Could you check a few things on this model? Use its own coordinates, in mm. A direction names the side the tool comes from. Give positions to 0.01 mm unless a question says otherwise; leave off trailing zeros. Order: outer loops, then holes, each group sorted by start corner. A loop starts at its lowest first (then second) coordinate and runs counter-clockwise, first axis right, second up. Notation, with made-up numbers: M 73,7.5 L 79,7.5 A15 ccw 79,25.5 Z; hole C 32,51.5 d6. An arc over 180 degrees is marked long. Use a Markdown table: item, result. Add a question column.
Item 1: Suppose I cut it at A-A on z = 28.5. Write out the boundary of the cut face in (x, y), plus the area to 3 significant figures.
Item 2: Suppose I cut it at B-B on x = 62. Count the separate pieces of the cut face and the enclosed holes in it, plus the area to 3 significant figures.
Item 3: If I drill on L1, parallel to Y at x = 60, z = 16; L2, parallel to X at y = 55.5, z = 36.5; L3, parallel to Y at x = 11.5, z = 43, over which ranges is the centre line in solid material (lowest first)? Write a range as from..to.
Item 4: If we mould it in two halves opening along X, with no side actions, what happens to faces 4 (the face through (2.85, 66.99, 5.07)), 5 (the face through (54.5, 65.1, 52.5)), 6 (the face through (65, 58, 55))? For each: released by +X, released by -X, zero draft, split by the parting line, or undercut.
Item 5: Suppose I cut it at C-C on x = 54. Write out the boundary of the cut face in (y, z), plus the area to 3 significant figures.
Item 6: I'm going to push flat-ended pins straight in: pin 1 Ø7.5 at (x, y) = (13, 11.5) entering from +Z; pin 2 Ø7.5 at (x, y) = (61, 9.5) entering from +Z; pin 3 Ø6 at (x, z) = (18.5, 53.5) entering from +Y; pin 4 Ø1.5 at (x, z) = (13, 33.5) entering from +Y. Where does each tip first touch, or does it pass through?
Item 7: For faces 1 (the face through (54.048, 5.436, 52.465)), 2 (the face through (27, 43, 40)), 3 (the face through (70, 35, 5)), which set-ups out of +Z, -Z, +X, -X, +Y, -Y let a thin tool reach every point of the face, with its end or its side?
from build123d import *

# Parameters (mm, degrees)
BASE_PLATE_SKETCH_W             = 70
BASE_PLATE_SKETCH_H             = 70
BASE_PLATE_DEPTH                = 10
CORNER_POSTS_SKETCH_R           = 7.5
CORNER_POSTS_4X_DEPTH           = 30
TOP_PLATE_SKETCH_W              = 70
TOP_PLATE_SKETCH_H              = 70
TOP_PLATE_DEPTH                 = 10
POST_BOSSES_SKETCH_R            = 7.5
POST_BOSSES_SKETCH_R_2          = 5
POST_BOSSES_4X_DEPTH            = 5
CENTRE_BOSS_SKETCH_R            = 15
CENTRE_BOSS_SKETCH_R_2          = 11
CENTRE_BOSS_30_DEPTH            = 20
CENTRE_BORE_SKETCH_R            = 11
CENTRE_BORE_CUT_DEPTH           = 111.905365064
POST_HOLES_SKETCH_R             = 5
POST_HOLES_4X_DEPTH             = 111.905365064
TOP_PLATE_CORNER_FILLETS_R10_R  = 10
BASE_PLATE_CORNER_FILLETS_R10_R = 10


with BuildPart() as part:
    # Base Plate Sketch → Base Plate (new body)
    with BuildSketch(Plane.XY):
        with Locations((35, 35)):
            Rectangle(BASE_PLATE_SKETCH_W, BASE_PLATE_SKETCH_H)
    extrude(amount=BASE_PLATE_DEPTH)

    # Corner Posts Sketch → Corner Posts 4x (add)
    with BuildSketch(Plane.XY.offset(10)):
        with Locations((10, 10)):
            Circle(CORNER_POSTS_SKETCH_R)
        with Locations((60, 10)):
            Circle(CORNER_POSTS_SKETCH_R)
        with Locations((60, 60)):
            Circle(CORNER_POSTS_SKETCH_R)
        with Locations((10, 60)):
            Circle(CORNER_POSTS_SKETCH_R)
    extrude(amount=CORNER_POSTS_4X_DEPTH)

    # Top Plate Sketch → Top Plate (add)
    with BuildSketch(Plane.XY.offset(40)):
        with Locations((35, 35)):
            Rectangle(TOP_PLATE_SKETCH_W, TOP_PLATE_SKETCH_H)
    extrude(amount=TOP_PLATE_DEPTH)

    # Post Bosses Sketch → Post Bosses 4x (add)
    # profile 1 of 4: a face of its own
    with BuildSketch(Plane.XY.offset(50)):
        with Locations((10, 60)):
            Circle(POST_BOSSES_SKETCH_R)
        with Locations((10, 60)):
            Circle(POST_BOSSES_SKETCH_R_2, mode=Mode.SUBTRACT)
    # profile 2 of 4: a face of its own
    with BuildSketch(Plane.XY.offset(50)):
        with Locations((60, 60)):
            Circle(POST_BOSSES_SKETCH_R)
        with Locations((60, 60)):
            Circle(POST_BOSSES_SKETCH_R_2, mode=Mode.SUBTRACT)
    # profile 3 of 4: a face of its own
    with BuildSketch(Plane.XY.offset(50)):
        with Locations((10, 10)):
            Circle(POST_BOSSES_SKETCH_R)
        with Locations((10, 10)):
            Circle(POST_BOSSES_SKETCH_R_2, mode=Mode.SUBTRACT)
    # profile 4 of 4: a face of its own
    with BuildSketch(Plane.XY.offset(50)):
        with Locations((60, 10)):
            Circle(POST_BOSSES_SKETCH_R)
        with Locations((60, 10)):
            Circle(POST_BOSSES_SKETCH_R_2, mode=Mode.SUBTRACT)
    extrude(amount=POST_BOSSES_4X_DEPTH)

    # Centre Boss Sketch → Centre Boss Ø30 (add)
    with BuildSketch(Plane.XY.offset(50)):
        with Locations(Location((35, 35, 0), (0, 0, 180))):
            Circle(CENTRE_BOSS_SKETCH_R)
        with Locations((35, 35)):
            Circle(CENTRE_BOSS_SKETCH_R_2, mode=Mode.SUBTRACT)
    extrude(amount=CENTRE_BOSS_30_DEPTH)

    # Centre Bore Sketch → Centre Bore Cut (cut, through all)
    with BuildSketch(Plane.XY.offset(50)):
        with Locations(Location((35, 35, 0), (0, 0, 180))):
            Circle(CENTRE_BORE_SKETCH_R)
    extrude(amount=-CENTRE_BORE_CUT_DEPTH, mode=Mode.SUBTRACT)

    # Post Holes Sketch → Post Holes 4x (cut, through all)
    with BuildSketch(Plane.XY.offset(50)):
        with Locations((60, 60)):
            Circle(POST_HOLES_SKETCH_R)
        with Locations((10, 60)):
            Circle(POST_HOLES_SKETCH_R)
        with Locations((60, 10)):
            Circle(POST_HOLES_SKETCH_R)
        with Locations((10, 10)):
            Circle(POST_HOLES_SKETCH_R)
    extrude(amount=-POST_HOLES_4X_DEPTH, mode=Mode.SUBTRACT)

    # Top Plate Corner Fillets R10
    top_plate_corner_fillets_r10_edges = [part.edges().sort_by_distance(p)[0] for p in [
        (0, 70, 45),
        (0, 0, 45),
        (70, 0, 45),
        (70, 70, 45),
    ]]
    fillet(top_plate_corner_fillets_r10_edges, radius=TOP_PLATE_CORNER_FILLETS_R10_R)

    # Base Plate Corner Fillets R10
    base_plate_corner_fillets_r10_edges = [part.edges().sort_by_distance(p)[0] for p in [
        (0, 70, 5),
        (70, 70, 5),
        (70, 0, 5),
        (0, 0, 5),
    ]]
    fillet(base_plate_corner_fillets_r10_edges, radius=BASE_PLATE_CORNER_FILLETS_R10_R)


solid = part.part
Findings below:
| question | item | result |
|---|---|---|
| 1 | outline | C 10,10 d15; C 10,60 d15; C 60,10 d15; C 60,60 d15; hole C 10,10 d10; hole C 10,60 d10; hole C 60,10 d10; hole C 60,60 d10 |
| 1 | area | 393 mm^2 |
| 2 | separate pieces | 3 |
| 2 | enclosed holes | 1 |
| 2 | area | 1,400 mm^2 |
| 3 | L1 | y = 2.5..5, 15..17.5, 52.5..55, 65..67.5 |
| 3 | L2 | x = 4..7.82, 12.18..16, 54..57.82, 62.18..66 |
| 3 | L3 | y = 0..5.23, 14.77..55.23, 64.77..70 |
| 4 | face 4 | released by -X |
| 4 | face 5 | undercut |
| 4 | face 6 | zero draft |
| 5 | outline | M 0,0 L 70,0 L 70,10 L 64.5,10 L 64.5,40 L 70,40 L 70,50 L 64.5,50 L 64.5,55 L 55.5,55 L 55.5,50 L 14.5,50 L 14.5,55 L 5.5,55 L 5.5,50 L 0,50 L 0,40 L 5.5,40 L 5.5,10 L 0,10 Z; hole M 14.5,10 L 55.5,10 L 55.5,40 L 14.5,40 Z |
| 5 | area | 2,030 mm^2 |
| 6 | pin 1 | stops at z = 55 |
| 6 | pin 2 | passes through |
| 6 | pin 3 | stops at y = 65.1 |
| 6 | pin 4 | stops at y = 67.15 |
| 7 | face 1 | +Z |
| 7 | face 2 | none |
| 7 | face 3 | +Z, -Z, +X, +Y, -Y |
